Source: CAD feature listing. Evaluate the final solid. Frame: model axes, mm. A direction names the side the tool comes from. Round coordinates to 2 decimals unless told otherwise and drop trailing zeros. Order: outer loops, then holes, each group sorted by start corner. A loop starts at its lowest first (then second) coordinate and runs counter-clockwise, first axis right, second up. Notation, with made-up numbers: (-21.75, 84) -> (23.25, 84) arc R22 cw to (23.25, 122) -> close; hole circle Ø6 at (19, -16). An arc over 180 degrees is marked (long way). Use a Markdown table: item, result. Add a question column.
```python
from build123d import *

# Parameters (mm, degrees)
SKETCH1_W           = 14
SKETCH1_H           = 5
SKETCH1_W_2         = 12
SKETCH1_H_2         = 3
BOSS_EXTRUDE1_DEPTH = 275
SKETCH2_W           = 29
SKETCH2_H           = 12
BOSS_EXTRUDE2_DEPTH = 1.5
SKETCH3_W           = 15
SKETCH3_H           = 12
BOSS_EXTRUDE3_DEPTH = 1.5
LPATTERN1_COUNT     = 2
LPATTERN1_PITCH     = 155
CHAMFER1_SIZE       = 1
CUT_EXTRUDE1_DEPTH  = 10
BOSS_EXTRUDE4_REACH = 279.078
FILLET1_R           = 3
BOSS_EXTRUDE5_REACH = 283.899
FILLET2_R           = 1
FILLET3_R           = 2


with BuildPart() as part:
    # Sketch1 → Boss-Extrude1 (new body)
    with BuildSketch(Plane(origin=(0, 0, 0), x_dir=(1, 0, 0), z_dir=(0, 1, 0))):
        Rectangle(SKETCH1_W, SKETCH1_H)
        Rectangle(SKETCH1_W_2, SKETCH1_H_2, mode=Mode.SUBTRACT)
    extrude(amount=BOSS_EXTRUDE1_DEPTH)

    # Sketch2 → Boss-Extrude2 (add)
    with BuildSketch(Plane(origin=(0, 0, -2.5), x_dir=(-1, 0, 0), z_dir=(0, 0, -1))):
        with Locations((7.5, 219)):
            Rectangle(SKETCH2_W, SKETCH2_H)
    boss_extrude2 = extrude(amount=BOSS_EXTRUDE2_DEPTH)

    # Sketch3 → Boss-Extrude3 (add)
    with BuildSketch(Plane.ZY.offset(22)):
        with Locations((-10, 219)):
            Rectangle(SKETCH3_W, SKETCH3_H)
    boss_extrude3 = extrude(amount=-BOSS_EXTRUDE3_DEPTH)

    # LPattern1: Boss-Extrude2, Boss-Extrude3 ×2
    with Locations(*[(0, -i * LPATTERN1_PITCH, 0) for i in range(1, LPATTERN1_COUNT)]):
        add(boss_extrude2)
        add(boss_extrude3)

    # Chamfer1
    chamfer1_edges = [part.edges().sort_by_distance(p)[0] for p in [
        (-21.25, 213, -17.5),
        (-21.25, 225, -17.5),
        (-21.25, 58, -17.5),
        (-21.25, 70, -17.5),
    ]]
    chamfer(chamfer1_edges, length=CHAMFER1_SIZE)

    # Sketch4 → Cut-Extrude1 (cut)
    with BuildSketch(Plane(origin=(-20.5, 0, 0), x_dir=(0, 0, -1), z_dir=(1, 0, 0))):
        with BuildLine():
            Line((8, 66), (14, 66))
            ThreePointArc((14, 66), (16, 64), (14, 62))
            Line((14, 62), (8, 62))
            ThreePointArc((8, 62), (6, 64), (8, 66))
        make_face()
        with BuildLine():
            Line((14, 217.25), (8, 217.25))
            ThreePointArc((8, 217.25), (6.25, 219), (8, 220.75))
            Line((8, 220.75), (14, 220.75))
            ThreePointArc((14, 220.75), (15.75, 219), (14, 217.25))
        make_face()
    extrude(amount=-CUT_EXTRUDE1_DEPTH, mode=Mode.SUBTRACT)

    # Boss-Extrude4: up to this face of the body (flat: up to its plane)
    boss_extrude4_end = Plane(part.part.faces().sort_by_distance((-7, 137.5, 0))[0])
    # Sketch5 → Boss-Extrude4 (add, up to the picked face)
    with BuildSketch(Plane(origin=(7, 0, 0), x_dir=(0, 0, -1), z_dir=(1, 0, 0)), mode=Mode.PRIVATE) as boss_extrude4_sk1:
        Polygon((-1.5, 275), (-3.55212086, 280.638155725), (-4.491813481, 280.296135581), (-1.5, 272.0761956), align=None)
    boss_extrude4_tool1 = split(extrude(boss_extrude4_sk1.sketch, amount=-BOSS_EXTRUDE4_REACH, mode=Mode.PRIVATE), bisect_by=boss_extrude4_end, keep=Keep.BOTH, mode=Mode.PRIVATE)
    boss_extrude4 = boss_extrude4_tool1.solids().sort_by(Axis((7, 276.951919, 2.775572), (-1, 0, 0)))[0]
    add(boss_extrude4)

    # Fillet1
    fillet1_edges = [part.edges().sort_by_distance(p)[0] for p in [
        (7, 280.467145653, 4.02196717),
        (-7, 280.467145653, 4.02196717),
    ]]
    fillet(fillet1_edges, radius=FILLET1_R)

    # Boss-Extrude5: up to this face of the body (flat: up to its plane)
    boss_extrude5_end = Plane(part.part.faces().sort_by_distance((0, 137.41183651, 2.5))[0])
    # Sketch6 → Boss-Extrude5 (add, up to the picked face)
    with BuildSketch(Plane(origin=(0, 0, -2.5), x_dir=(-1, 0, 0), z_dir=(0, 0, -1)), mode=Mode.PRIVATE) as boss_extrude5_sk1:
        Polygon((-6, 275), (-7.953408927, 280.673111454), (-8.898927502, 280.347543299), (-6, 271.928446513), align=None)
    boss_extrude5_tool1 = split(extrude(boss_extrude5_sk1.sketch, amount=-BOSS_EXTRUDE5_REACH, mode=Mode.PRIVATE), bisect_by=boss_extrude5_end, keep=Keep.BOTH, mode=Mode.PRIVATE)
    # Sketch6 → Boss-Extrude5 (add, up to the picked face)
    with BuildSketch(Plane(origin=(0, 0, -2.5), x_dir=(-1, 0, 0), z_dir=(0, 0, -1)), mode=Mode.PRIVATE) as boss_extrude5_sk2:
        Polygon((6, 275), (6, 271.928446513), (8.898927502, 280.347543299), (7.953408927, 280.673111454), align=None)
    boss_extrude5_tool2 = split(extrude(boss_extrude5_sk2.sketch, amount=-BOSS_EXTRUDE5_REACH, mode=Mode.PRIVATE), bisect_by=boss_extrude5_end, keep=Keep.BOTH, mode=Mode.PRIVATE)
    add(boss_extrude5_tool1.solids().sort_by(Axis((7.228438, 276.932112, -2.5), (0, 0, 1)))[0])
    add(boss_extrude5_tool2.solids().sort_by(Axis((-7.228438, 276.932112, -2.5), (0, 0, 1)))[0])

    # Fillet2
    fillet2_edges = [part.edges().sort_by_distance(p)[0] for p in [
        (8.426168215, 280.510327376, 2.5),
        (8.426168215, 280.510327376, -2.5),
        (-8.426168215, 280.510327376, 2.5),
        (-8.426168215, 280.510327376, -2.5),
    ]]
    fillet(fillet2_edges, radius=FILLET2_R)

    # Mirror1: Boss-Extrude4 across plane
    add(boss_extrude4.mirror(Plane.XY))

    # Fillet3
    fillet3_edges = [part.edges().sort_by_distance(p)[0] for p in [
        (-7, 280.467145653, -4.02196717),
        (7, 280.467145653, -4.02196717),
    ]]
    fillet(fillet3_edges, radius=FILLET3_R)


solid = part.part
```
1) Draft query along Z for faces 1 (the flat face through (0, 29, -2.5)), 2 (the flat face through (0.1, 277.6, 3.51)), 3 (the flat face through (0.1, 277.78, -2.51)). Return one class per face: pulls with the +Z half, pulls with the -Z half, needs draft (parallel to the pull), parting line crosses it, or undercut.
2) First-contact query: pin 1 Ø5 at (x, z) = (-4.5, 1.5) entering from -Y; pin 2 Ø2.5 at (y, z) = (105, 0.5) entering from +X; pin 3 Ø1.8 at (x, y) = (8, 276.5) entering from -Z; pin 4 Ø0.8 at (x, z) = (-21.5, -12) entering from +Y. Flat tips, straight axial feed; report the tip coordinate or a pass-through.
3) Line query: probe 1 along Z at (x, y) = (3.5, 124); probe 2 along Z at (x, y) = (-0.5, 219.5); probe 3 along X at (y, z) = (60, 1.75). Output: solid intervals per line, ascending. Write a range as from..to.
4) Section B-B on x = -14. Output: boundary loops of the cut face in (y, z).
5) Section A-A on y = 51. Output: boundary loops of the cut face in (x, z), then the cut area to 3 significant figures.
6) Reachability of faces 4 (the flat face through (-10.8, 70, -3.8)), 5 (the flat face through (0, 136, 1.5)), 6 (the flat face through (-7, 277.9, 0)), 7 (the flat face through (0, 135, 2.5)) from +Z, -Z, +X, -X, +Y, -Y: full face, straight path, thin tool, end or side. Return the list, or none.
Conclusion:
| question | item | result |
|---|---|---|
| 1 | face 1 | pulls with the -Z half |
| 1 | face 2 | pulls with the +Z half |
| 1 | face 3 | undercut |
| 2 | pin 1 | stops at y = 0 |
| 2 | pin 2 | stops at x = 7 |
| 2 | pin 3 | stops at z = -2.5 |
| 2 | pin 4 | stops at y = 225 |
| 3 | probe 1 | z = -2.5..-1.5, 1.5..2.5 |
| 3 | probe 2 | z = -4..-1.5, 1.5..2.5 |
| 3 | probe 3 | x = -7..7 |
| 4 | outline | (58, -4) -> (70, -4) -> (70, -2.5) -> (58, -2.5) -> close; (213, -4) -> (225, -4) -> (225, -2.5) -> (213, -2.5) -> close |
| 5 | outline | (-7, -2.5) -> (7, -2.5) -> (7, 2.5) -> (-7, 2.5) -> close; hole (-6, -1.5) -> (6, -1.5) -> (6, 1.5) -> (-6, 1.5) -> close |
| 5 | area | 34.0 mm^2 |
| 6 | face 4 | -Z, +X, -X |
| 6 | face 5 | +Y, -Y |
| 6 | face 6 | +Y |
| 6 | face 7 | +Z, +X, -X, -Y |
